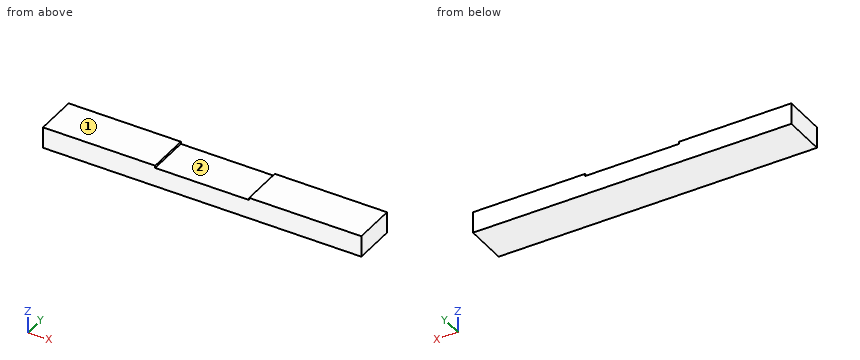
```python
from build123d import *

# Parameters (mm, degrees)
SKETCH_1_W          = 210
SKETCH_1_H          = 28
EXTRUDE_1_DEPTH     = 14
SKETCH_2_W          = 62
SKETCH_2_H          = 28
CUT_EXTRUDE_1_DEPTH = 1.5


with BuildPart() as part:
    # 草图1 → 凸台-拉伸1 (new body)
    with BuildSketch(Plane.XY):
        Rectangle(SKETCH_1_W, SKETCH_1_H)
    extrude(amount=EXTRUDE_1_DEPTH)

    # 草图2 → 切除-拉伸1 (cut)
    with BuildSketch(Plane.XY.offset(14)):
        Rectangle(SKETCH_2_W, SKETCH_2_H)
    extrude(amount=-CUT_EXTRUDE_1_DEPTH, mode=Mode.SUBTRACT)


solid = part.part
```
Build history of the part. All positions in model axes, mm. Face numbers are marked on the shaded views. Coordinates: 2 decimals unless noted, no trailing zeros. Order: outer loops, then holes, each group sorted by start corner. A loop starts at its lowest first (then second) coordinate and runs counter-clockwise, first axis right, second up. Notation, with made-up numbers: (61, 16.5) -> (68, 16.5) arc R21 cw to (68, 39.5) -> close; hole circle Ø2 at (83, 83). An arc over 180 degrees is marked (long way). Answer in a Markdown table with one row per item. Add a question column.
Q1. Band-saw the part on B-B, the plane x = -9. List the corners of the cut face in (y, z), then the cut area to 3 significant figures.
Q2. Band-saw the part on A-A, the plane y = 4.5. List the corners of the cut face in (x, z).
Q3. Mould opens along X. For the marked faces 1 and 2 say: +X half, -X half, draft (parallel to the pull), parting line (faces both ways), or undercut.
Q4. Wall check: line 1 along Z through (x, y) = (19, -12.75). Give the ranges that are in metal, low to high. Write a range as [from, to].
Q5. Drop flat-ended pins along their axis: pin 1 (14 mm diameter, centred on x = -4.5, y = -5.5, fed in from +Z); pin 2 (2 mm diameter, centred on x = 57, y = 8.5, fed in from -Z). Give the stop position or say it passes through.
Answers follow:
| question | item | result |
|---|---|---|
| 1 | outline | (-14, 0) -> (14, 0) -> (14, 12.5) -> (-14, 12.5) -> close |
| 1 | area | 350 mm^2 |
| 2 | outline | (-105, 0) -> (105, 0) -> (105, 14) -> (31, 14) -> (31, 12.5) -> (-31, 12.5) -> (-31, 14) -> (-105, 14) -> close |
| 3 | face 1 | draft |
| 3 | face 2 | undercut |
| 4 | line 1 | [0, 12.5] |
| 5 | pin 1 | z = 12.5 |
| 5 | pin 2 | z = 0 |
